Can you work these out from the drawing? Everything is in mm from the part's minimum corner. A direction names the side the tool comes from. Round coordinates to 2 decimals unless told otherwise and drop trailing zeros. Order: outer loops, then holes, each group sorted by start corner. A loop starts at its lowest first (then second) coordinate and runs counter-clockwise, first axis right, second up. Notation, with made-up numbers: M 84.25,33 L 102.25,33 A6 cw 102.25,41 Z; hole C 22.5,72.25 d6. An arc over 180 degrees is marked long. Write item = value, one per line. Start each with the question number.
Item 1: We'd pull the mould along X, two halves only. Please class the marked faces 1, 2 and 3: pulls with the +X half, pulls with the -X half, needs draft (parallel to the pull), parting line crosses it, or undercut.
Item 2: I want a section at A-A, the plane y = 10. List the corners of the cut face in (x, z) for me (1 decimal).
Item 3: I want a section at B-B, the plane x = 15. List the corners of the cut face in (y, z) for me (1 decimal).
Item 4: Please list where these lines run through material, in increasing order: L1, parallel to Y at x = 15, z = 1.75 (1 decimal); L2, parallel to Z at x = 104, y = 35; L3, parallel to X at y = 22.5, z = 26.5 (1 decimal).
Item 5: I want a section at C-C, the plane y = 20.5. List the corners of the cut face in (x, z) for me.
Item 6: I want a section at D-D, the plane x = 55. List the corners of the cut face in (y, z) for me.
Item 7: I'm going to push flat-ended pins straight in: P1, Ø1, axis at x = 34.5, y = 12.5, coming from the -Z side; P2, Ø11, axis at x = 101.5, y = 27, coming from the +Z side; P3, Ø8, axis at y = 19.5, z = 16, coming from the -X side. Where does each tip first touch, or does it pass through?
Item 8: For the marked faces 4, 5, 6 and 7, which set-ups out of +Z, -Z, +X, -X, +Y, -Y let a thin tool reach every point of the face, with its end or its side?
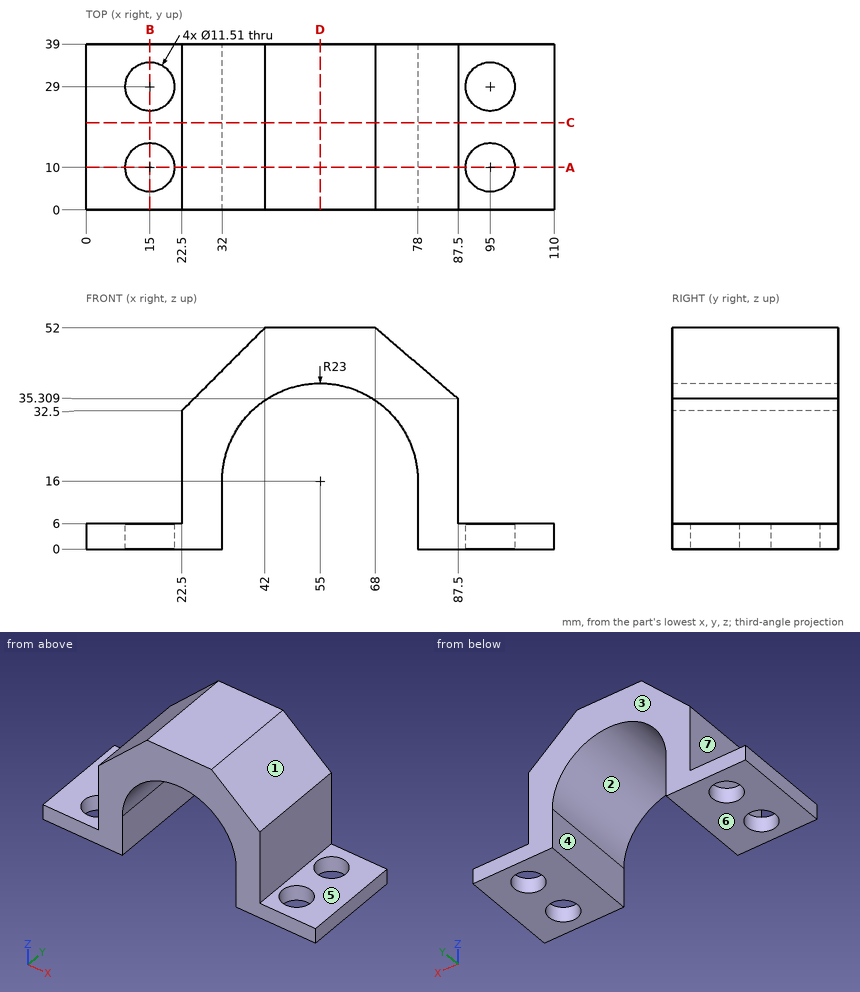
Filled in:
q1.face_1 = pulls with the +X half
q1.face_2 = undercut
q1.face_3 = needs draft
q2.outline = M 0,0 L 9.2,0 L 9.2,6 L 0,6 Z; M 20.8,0 L 32,0 L 32,16 A23 cw 78,16 L 78,0 L 89.2,0 L 89.2,6 L 87.5,6 L 87.5,35.3 L 68,52 L 42,52 L 22.5,32.5 L 22.5,6 L 20.8,6 Z; M 100.8,0 L 110,0 L 110,6 L 100.8,6 Z
q3.outline = M 0,0 L 4.2,0 L 4.2,6 L 0,6 Z; M 15.8,0 L 23.2,0 L 23.2,6 L 15.8,6 Z; M 34.8,0 L 39,0 L 39,6 L 34.8,6 Z
q4.L1 = 0 to 4.2, 15.8 to 23.2, 34.8 to 39
q4.L2 = 0 to 6
q4.L3 = 22.5 to 34.5, 75.5 to 87.5
q5.outline = M 0,0 L 32,0 L 32,16 A23 cw 78,16 L 78,0 L 110,0 L 110,6 L 87.5,6 L 87.5,35.31 L 68,52 L 42,52 L 22.5,32.5 L 22.5,6 L 0,6 Z
q6.outline = M 0,39 L 39,39 L 39,52 L 0,52 Z
q7.P1 = 25.38
q7.P2 = 6
q7.P3 = 22.5
q8.face_4 = -Z, +Y, -Y
q8.face_5 = +Z, +X, +Y, -Y
q8.face_6 = -Z, +X, -X, +Y, -Y
q8.face_7 = +Z, -X, +Y, -Y
